Can you work these out from the model? Positions are in its coordinate system, mm. Face numbers are marked on the shaded views. A direction names the side the tool comes from. Give positions to 0.01 mm unless a question says otherwise; leave off trailing zeros. Order: outer loops, then holes, each group sorted by start corner. A loop starts at its lowest first (then second) coordinate and runs counter-clockwise, first axis right, second up. Notation, with made-up numbers: (-33, -20.75) - (-9, -20.75) arc R21 cw to (-9, 2.25) - close; hole circle Ø3 at (80, 23). An arc over 180 degrees is marked (long way). One line per question, with ' | ' between items.
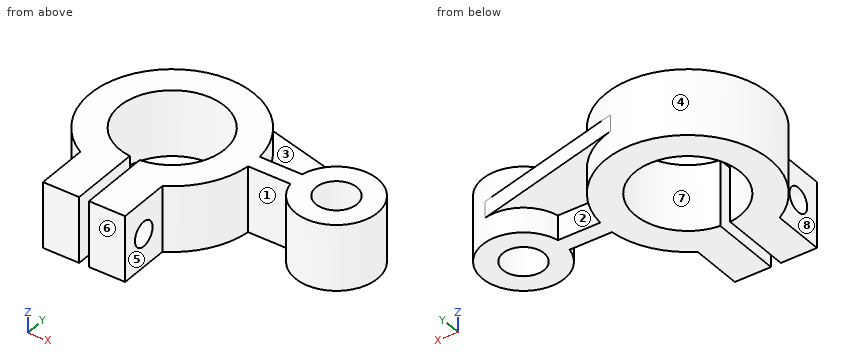
```python
from build123d import *

# Parameters (mm, degrees)
CLAMP_RING_SKETCH_R                       = 50
CLAMP_RING_SKETCH_R_2                     = 32
CLAMP_RING_100_BORE_64_DEPTH              = 20
CLAMP_BLOCK_AND_SECONDARY_BOSS_SKETCH_R   = 25
CLAMP_BLOCK_AND_SECONDARY_BOSS_SKETCH_R_2 = 12.5
CLAMP_BLOCK_AND_SECONDARY_BOSS_SKETCH_W   = 50
CLAMP_BLOCK_AND_SECONDARY_BOSS_SKETCH_H   = 31.698729811
CLAMP_BLOCK_AND_SECONDARY_BOSS_DEPTH      = 20
CLAMP_SLOT_6MM_DEPTH                      = 148.139389696
CLAMP_SLOT_6MM_DEPTH_BACK                 = 148.139389696
CLAMP_SLOT_SKETCH_W                       = 6
CLAMP_SLOT_SKETCH_H                       = 43.140935356
CONNECTING_WEB_SKETCH_W                   = 55.5
CONNECTING_WEB_SKETCH_H                   = 10
CONNECTING_WEB_10MM_DEPTH                 = 20
STIFFENING_RIB_10MM_REACH                 = 149.139
STIFFENING_RIB_SKETCH_WALL_W              = 393.103363046
STIFFENING_RIB_SKETCH_WALL_H              = 10
CLAMP_BOLT_HOLE_15_DEPTH                  = 148.139389696
CLAMP_BOLT_HOLE_15_DEPTH_BACK             = 148.139389696
CLAMP_BOLT_HOLE_SKETCH_R                  = 7.5


with BuildPart() as part:
    # Clamp Ring Sketch → Clamp Ring Ø100 Bore Ø64 (new, symmetric)
    with BuildSketch(Plane.XY):
        Circle(CLAMP_RING_SKETCH_R)
        Circle(CLAMP_RING_SKETCH_R_2, mode=Mode.SUBTRACT)
    extrude(amount=CLAMP_RING_100_BORE_64_DEPTH, both=True)

    # Clamp Block and Secondary Boss Sketch → Clamp Block and Secondary Boss (add, symmetric)
    # profile 1 of 2: a face of its own
    with BuildSketch(Plane.XY):
        with Locations((100, 0)):
            Circle(CLAMP_BLOCK_AND_SECONDARY_BOSS_SKETCH_R)
        with Locations((100, 0)):
            Circle(CLAMP_BLOCK_AND_SECONDARY_BOSS_SKETCH_R_2, mode=Mode.SUBTRACT)
    # profile 2 of 2: a face of its own
    with BuildSketch(Plane.XY):
        with Locations((0, -59.150635095)):
            Rectangle(CLAMP_BLOCK_AND_SECONDARY_BOSS_SKETCH_W, CLAMP_BLOCK_AND_SECONDARY_BOSS_SKETCH_H)
    extrude(amount=CLAMP_BLOCK_AND_SECONDARY_BOSS_DEPTH, both=True)


with BuildPart() as clamp_block_and_secondary_boss_piece_1:
    # of the separate pieces the step leaves, piece 1, a body of its own (clamp_block_and_secondary_boss_pieces)
    add(part.part.solids().sort_by_distance((-25, -43.301270189, 20))[0])

    # Clamp Slot Sketch → Clamp Slot 6mm (cut, two sides: drawn at the far end of the back side and taken through both)
    with BuildSketch(Plane.XY.offset(-CLAMP_SLOT_6MM_DEPTH_BACK)):
        with Locations((0, -53.429532322)):
            Rectangle(CLAMP_SLOT_SKETCH_W, CLAMP_SLOT_SKETCH_H)
    extrude(amount=CLAMP_SLOT_6MM_DEPTH + CLAMP_SLOT_6MM_DEPTH_BACK, mode=Mode.SUBTRACT)



with BuildPart() as clamp_block_and_secondary_boss_piece_2:
    # of the separate pieces the step leaves, piece 2, a body of its own (clamp_block_and_secondary_boss_pieces)
    add(part.part.solids().sort_by_distance((125, 0, -20))[0])


with BuildPart() as clamp_block_and_secondary_boss_piece_1_1:
    add(clamp_block_and_secondary_boss_piece_1.part)

    add(clamp_block_and_secondary_boss_piece_2.part)  # Connecting Web 10mm merges Clamp Block and Secondary Boss piece 2
    # Connecting Web Sketch → Connecting Web 10mm (add, symmetric)
    with BuildSketch(Plane.XY):
        with Locations((59.75, 0)):
            Rectangle(CONNECTING_WEB_SKETCH_W, CONNECTING_WEB_SKETCH_H)
    extrude(amount=CONNECTING_WEB_10MM_DEPTH, both=True)

    # Stiffening Rib Sketch wall → Stiffening Rib 10mm (add, up to next)
    with BuildSketch(Plane(origin=(59.375, 36.309218871, 0), x_dir=(-0.968245836551, 0.250000000002, 0), z_dir=(-0.250000000002, -0.968245836551, 0)), mode=Mode.PRIVATE) as stiffening_rib_10mm_sk1:
        Rectangle(STIFFENING_RIB_SKETCH_WALL_W, STIFFENING_RIB_SKETCH_WALL_H)
    stiffening_rib_10mm_tool1 = extrude(stiffening_rib_10mm_sk1.sketch, amount=STIFFENING_RIB_10MM_REACH, mode=Mode.PRIVATE) - clamp_block_and_secondary_boss_piece_1_1.part
    add(stiffening_rib_10mm_tool1.solids().sort_by_distance((59.375, 36.309218871, 0))[0])

    # Clamp Bolt Hole Sketch → Clamp Bolt Hole Ø15 (cut, two sides: drawn at the far end of the back side and taken through both)
    with BuildSketch(Plane(origin=(0, 0, 0), x_dir=(0, 0, -1), z_dir=(1, 0, 0)).offset(-CLAMP_BOLT_HOLE_15_DEPTH_BACK)):
        with Locations(Location((0, -59.150635095, 0), (0, 0, 270))):
            Circle(CLAMP_BOLT_HOLE_SKETCH_R)
    extrude(amount=CLAMP_BOLT_HOLE_15_DEPTH + CLAMP_BOLT_HOLE_15_DEPTH_BACK, mode=Mode.SUBTRACT)


solid = clamp_block_and_secondary_boss_piece_1_1.part
```
(1) Imagine slicing it at C-C (z = 16.5). List the corners of the cut face in (x, y) for me.
Answer below:
outline: (-25, -75) - (-3, -75) - (-3, -31.86) arc R32 cw (long way) to (3, -31.86) - (3, -75) - (25, -75) - (25, -43.3) arc R50 ccw to (49.75, -5) - (75.51, -5) arc R25 ccw (long way) to (75.51, 5) - (49.75, 5) arc R50 ccw (long way) to (-25, -43.3) - close; hole circle Ø25 at (100, 0)
(2) On a 3-axis mill with a long thin cutter (end or side, diameter ignored), from which of +Z, -Z, +X, -X, +Y, -Y can I reach the whole of each face in a straight line? I mean the marked faces 1, 2, 3, 4 and 5. Say none if no direction works.
Answer below:
face 1: +Z, -Z, -Y | face 2: -Z, +Y | face 3: +Z, +Y | face 4: none | face 5: +Z, -Z, +X, -Y
(3) Imagine slicing it at D-D (x = 7). List the corners of the cut face in (y, z) for me.
Answer below:
outline: (-75, -20) - (-31.22, -20) - (-31.22, 20) - (-75, 20) - close; (31.22, -20) - (49.51, -20) - (49.51, 20) - (31.22, 20) - close; hole circle Ø15 at (-59.15, 0)
(4) Will these pins go through, and if not, where does the flat tip stop? pin 1 (20 mm diameter, centred on y = -56.5, z = -8, fed in from -X); pin 2 (13 mm diameter, centred on x = 74, y = 19.5, fed in from -Z); pin 3 (4.5 mm diameter, centred on x = 64.5, z = -9, fed in from +Y); pin 4 (10 mm diameter, centred on x = -3.5, z = -6, fed in from +Y).
Answer below:
pin 1: x = -25 | pin 2: z = -5 | pin 3: y = 5 | pin 4: y = 50
(5) If we mould it in two halves opening along X, with no side actions, what happens to the marked faces 6, 7 and 8? For each: released by +X, released by -X, zero draft, split by the parting line, or undercut.
Answer below:
face 6: zero draft | face 7: undercut | face 8: released by -X
(6) If I drill on line 1 (X direction, y = 22, z = -13.5); line 2 (X direction, y = -69, z = -16.5); line 3 (X direction, y = 6, z = 4), over which ranges is the centre line in solid material (lowest first)?
Answer below:
line 1: -44.9 to -23.24, 23.24 to 44.9, 88.13 to 111.87 | line 2: -25 to -3, 3 to 25 | line 3: -49.64 to -31.43, 31.43 to 89.03, 110.97 to 124.27
(7) Imagine slicing it at B-B (y = 0). List the corners of the cut face in (x, z) for me, and give its area (3 significant figures).
Answer below:
outline: (-50, -20) - (-32, -20) - (-32, 20) - (-50, 20) - close; (32, -20) - (87.5, -20) - (87.5, 20) - (32, 20) - close; (112.5, -20) - (125, -20) - (125, 20) - (112.5, 20) - close | area: 3,440 mm^2
(8) Imagine slicing it at A-A (z = 0). List the corners of the cut face in (x, y) for me, and give its area (3 significant figures).
Answer below:
outline: (-25, -75) - (-3, -75) - (-3, -66.65) - (-25, -66.65) - close; (-25, -51.65) - (-3, -51.65) - (-3, -31.86) arc R32 cw (long way) to (3, -31.86) - (3, -51.65) - (25, -51.65) - (25, -43.3) arc R50 ccw to (49.75, -5) - (75.51, -5) arc R25 ccw (long way) to (106.25, 24.21) - (12.5, 48.41) arc R50 ccw to (-25, -43.3) - close; (3, -75) - (25, -75) - (25, -66.65) - (3, -66.65) - close; hole circle Ø25 at (100, 0) | area: 8,090 mm^2
